```python
from build123d import *

# Parameters (mm, degrees)
SKETCH1_R           = 20
BOSS_EXTRUDE1_DEPTH = 1
SKETCH2_R           = 2
BOSS_EXTRUDE2_DEPTH = 1
SKETCH3_R           = 12.5
BOSS_EXTRUDE3_DEPTH = 1


with BuildPart() as part:
    # Sketch1 → Boss-Extrude1 (new body)
    with BuildSketch(Plane.XY):
        Circle(SKETCH1_R)
    extrude(amount=BOSS_EXTRUDE1_DEPTH)

    # Sketch2 → Boss-Extrude2 (add)
    with BuildSketch(Plane(origin=(0, 0, 0), x_dir=(-1, 0, 0), z_dir=(0, 0, -1))):
        with Locations(Location((0, 0, 0), (0, 0, 180))):
            Circle(SKETCH2_R)
    extrude(amount=BOSS_EXTRUDE2_DEPTH)

    # Sketch3 → Boss-Extrude3 (add)
    with BuildSketch(Plane(origin=(0, 0, -1), x_dir=(-1, 0, 0), z_dir=(0, 0, -1))):
        Circle(SKETCH3_R)
    extrude(amount=BOSS_EXTRUDE3_DEPTH)


solid = part.part
```
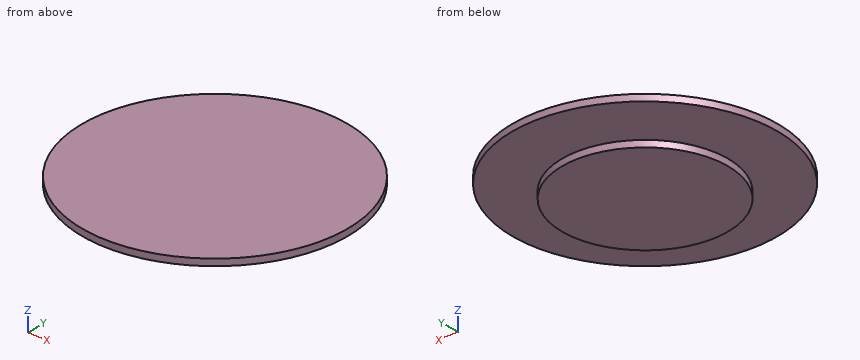
The listing builds one solid part. Answer for the finished solid, in the listing's coordinates (mm). Give positions to 0.01 mm unless a question says otherwise; leave off trailing zeros. Write each loop counter-clockwise with the first axis right and the second up, starting at its lowest first coordinate (ties: lowest second). Pieces come first, ordered by that corner, then holes. Notation, with made-up numbers: (32, -28.5) -> (81, -28.5) arc R11 ccw to (81, -11.5) -> close; hole circle Ø6 at (60, 3.5). An arc over 180 degrees is marked (long way). Write item = value, one per line. Start each with the question number.
1) Each of these flat-tipped pins is pushed along its axis until it touches: pin 1 (1.5 mm diameter, centred on x = -1.5, z = 0, fed in from -Y); pin 2 (1 mm diameter, centred on x = -3.5, z = -1.5, fed in from +Y); pin 3 (1 mm diameter, centred on x = -6.5, z = 0, fed in from +Y). Where does it stop, or does it pass through?
2) Straight lines are drawn through the part: line 1 along Z through (x, y) = (7, 5.5); line 2 along Z through (x, y) = (7, -13); line 3 along Y through (x, z) = (0.5, -1.8). For each, find the intervals that lie inside material, in ascending order.
3) The part is cut by section C-C, the plane y = 0. Determine the outline of the cut face in (x, z), and give its area (3 significant figures).
4) The part is cut by section A-A, the plane y = -4. Determine the outline of the cut face in (x, z).
5) The part is cut by section B-B, the plane x = -11.5. Determine the outline of the cut face in (y, z), and give its area (3 significant figures).
Solutions:
q1.pin_1 = -19.99
q1.pin_2 = 12.13
q1.pin_3 = 19.08
q2.line_1 = -2 to -1, 0 to 1
q2.line_2 = 0 to 1
q2.line_3 = -12.49 to 12.49
q3.outline = (-20, 0) -> (-2, 0) -> (-2, -1) -> (-12.5, -1) -> (-12.5, -2) -> (12.5, -2) -> (12.5, -1) -> (2, -1) -> (2, 0) -> (20, 0) -> (20, 1) -> (-20, 1) -> close
q3.area = 69.0 mm²
q4.outline = (-19.6, 0) -> (19.6, 0) -> (19.6, 1) -> (-19.6, 1) -> close; (-11.84, -2) -> (11.84, -2) -> (11.84, -1) -> (-11.84, -1) -> close
q5.outline = (-16.36, 0) -> (16.36, 0) -> (16.36, 1) -> (-16.36, 1) -> close; (-4.9, -2) -> (4.9, -2) -> (4.9, -1) -> (-4.9, -1) -> close
q5.area = 42.5 mm²
